```python
from build123d import *

# Parameters (mm, degrees)
SKETCH1_R             = 7.5
BOSS_EXTRUDE1_DEPTH   = 15
SKETCH2_W             = 130
SKETCH2_H             = 40
BOSS_EXTRUDE2_DEPTH   = 3
M8_TAPPED_HOLE1_D     = 6.8
M8_TAPPED_HOLE1_DEPTH = 19.75
M8_TAPPED_HOLE1_TIP   = 2.042926105
CHAMFER1_SIZE         = 1


with BuildPart() as part:
    # Sketch1 → Boss-Extrude1 (new body)
    with BuildSketch(Plane(origin=(0, 0, 0), x_dir=(1, 0, 0), z_dir=(0, 1, 0))):
        with Locations(Location((0, 0, 0), (0, 0, 270))):
            Circle(SKETCH1_R)
    extrude(amount=BOSS_EXTRUDE1_DEPTH)

    # Sketch2 → Boss-Extrude2 (add)
    with BuildSketch(Plane(origin=(0, 15, 0), x_dir=(1, 0, 0), z_dir=(0, 1, 0))):
        Rectangle(SKETCH2_W, SKETCH2_H)
    extrude(amount=BOSS_EXTRUDE2_DEPTH)

    # M8 Tapped Hole1
    with Locations(Plane(origin=(0, 0, 0), x_dir=(-1, 0, 0), z_dir=(0, -1, 0))):
        with Locations((0, 0)):
            Hole(M8_TAPPED_HOLE1_D / 2, depth=M8_TAPPED_HOLE1_DEPTH)
            with Locations((0, 0, -(M8_TAPPED_HOLE1_DEPTH + M8_TAPPED_HOLE1_TIP / 2))):  # 118° drill point
                Cone(0, M8_TAPPED_HOLE1_D / 2, M8_TAPPED_HOLE1_TIP, mode=Mode.SUBTRACT)

    # Chamfer1
    chamfer1_edges = [part.edges().sort_by_distance(p)[0] for p in [
        (0, 0, -7.5),
        (0, 15, -7.5),
        (65, 16.5, 20),
        (65, 16.5, -20),
        (-65, 16.5, -20),
        (-65, 16.5, 20),
    ]]
    chamfer(chamfer1_edges, length=CHAMFER1_SIZE)


solid = part.part
```
The listing builds one solid part. Answer for the finished solid, in the listing's coordinates (mm). Coordinates: 2 decimals unless noted, no trailing zeros. Loops run counter-clockwise (first coordinate to the right, second up) from the corner with the lowest first, then second, coordinate; pieces in that order, holes last. Notation, with made-up numbers: M 12,87.5 L 33,87.5 A11 ccw 33,92.5 Z; hole C 51,69.5 d11. An arc over 180 degrees is marked long. Answer as a JSON object with one key per item and string values. Group by question number.
Item 1: Each of these flat-tipped pins is pushed along its axis until it touches: P1, Ø2, axis at y = 9.5, z = 1.5, coming from the -X side; P2, Ø3, axis at y = 2.5, z = 1, coming from the +X side; P3, Ø20, axis at x = -32.5, z = 0, coming from the -Y side. Where does it stop, or does it pass through?
Item 2: Section D-D (y = 10) is taken. Write down the section's boundary in (x, z).
Item 3: Section B-B (z = 0) is taken. Write down the section's boundary in (x, y), and give its area (3 significant figures).
Item 4: Consider L1, parallel to Y at x = -36, z = 3.5; L2, parallel to X at y = 1, z = -0.5; L3, parallel to X at y = 2.75, z = 5.5. Determine where each line is inside the solid, lowest interval first.
Item 5: Determine the mould class of faces 1 (the face through (-0.74, 9.13, 3.32)), 2 (the face through (-1, 18, -5)), 3 (the face through (-65, 16, 0)), 4 (the face through (0.33, 7.409, -7.493)) for opening direction X: +X half, -X half, draft (parallel to the pull), parting line (faces both ways), or undercut.
Item 6: Section A-A (x = 0) is taken. Write down the section's boundary in (y, z), and give its area (3 significant figures).
Item 7: Section C-C (x = -19) is taken. Write down the section's boundary in (y, z), and give its area (3 significant figures).
Solved:
{
 "1": {"P1": "stops at x = -7.48", "P2": "stops at x = 7.5", "P3": "stops at y = 15"},
 "2": {"outline": "C 0,0 d15; hole C 0,0 d6.8"},
 "3": {"outline": "M -65,15 L -8.5,15 L -7.5,14 L -7.5,1 L -6.5,0 L -3.4,0 L -3.4,18 L -65,18 Z; M 3.4,0 L 6.5,0 L 7.5,1 L 7.5,14 L 8.5,15 L 65,15 L 65,18 L 3.4,18 Z", "area": "493 mm2"},
 "4": {"L1": "y = 15 to 18", "L2": "x = -7.48 to -3.36, 3.36 to 7.48", "L3": "x = -5.1 to 5.1"},
 "5": {"face 1": "undercut", "face 2": "draft", "face 3": "-X half", "face 4": "parting line"},
 "6": {"outline": "M 0,-6.5 L 1,-7.5 L 14,-7.5 L 15,-8.5 L 15,-20 L 18,-20 L 18,-3.4 L 0,-3.4 Z; M 0,3.4 L 18,3.4 L 18,20 L 15,20 L 15,8.5 L 14,7.5 L 1,7.5 L 0,6.5 Z", "area": "223 mm2"},
 "7": {"outline": "M 15,-20 L 18,-20 L 18,20 L 15,20 Z", "area": "120 mm2"}
}
